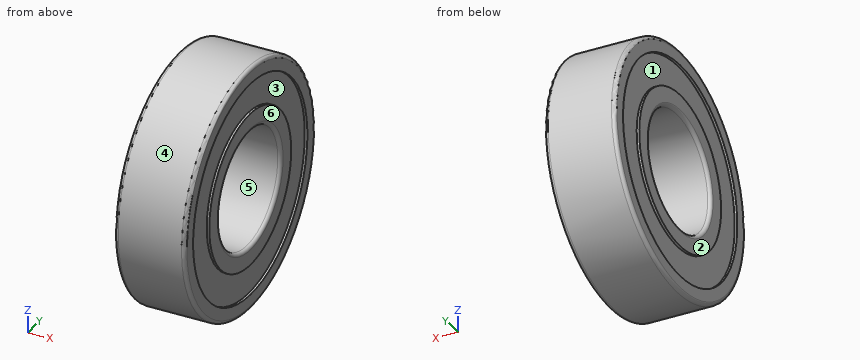
```python
from build123d import *


with BuildPart() as part:
    # 草图1 → 旋转1 (revolve)
    with BuildSketch(Plane.XY, mode=Mode.PRIVATE) as revolve_1_sk:
        with BuildLine():
            Line((0, 20.4), (0, 18.4))
            Line((0, 18.4), (0.433, 18.4))
            Line((0.433, 18.4), (0.433, 13.2))
            Line((0.433, 13.2), (0, 13.2))
            Line((0, 13.2), (0, 10.6))
            ThreePointArc((0, 10.6), (0.175735931, 10.175735931), (0.6, 10))
            Line((0.6, 10), (11.4, 10))
            ThreePointArc((11.4, 10), (11.824264069, 10.175735931), (12, 10.6))
            Line((12, 10.6), (12, 13.2))
            Line((12, 13.2), (11.567, 13.2))
            Line((11.567, 13.2), (11.567, 18.4))
            Line((11.567, 18.4), (12, 18.4))
            Line((12, 18.4), (12, 20.4))
            ThreePointArc((12, 20.4), (11.824264069, 20.824264069), (11.4, 21))
            Line((11.4, 21), (0.6, 21))
            ThreePointArc((0.6, 21), (0.175735931, 20.824264069), (0, 20.4))
        make_face()
    revolve(revolve_1_sk.sketch.rotate(Axis((12, 0, 0), (-1, 0, 0)), 270), axis=Axis((12, 0, 0), (-1, 0, 0)))


solid = part.part
```
Input: part model. Units: mm. Frame: model coordinates. Face numbers are marked on the shaded views. A direction names the side the tool comes from. Coordinates: 2 decimals unless noted, no trailing zeros. Order: outer loops, then holes, each group sorted by start corner. A loop starts at its lowest first (then second) coordinate and runs counter-clockwise, first axis right, second up. Notation, with made-up numbers: (33, -27) - (49, -27) arc R23 ccw to (49, -17) - close; hole circle Ø7 at (-18, 18). An arc over 180 degrees is marked (long way). Return JSON: item names as keys, results as strings.
Q1. Cut plane C-C (x = 5). Return loops of the section in (y, z).
The answers:
{"outline": "circle Ø42 at (0, 0); hole circle Ø20 at (0, 0)"}
Q2. First-contact query: pin 1 (1.5 mm diameter, centred on x = 10.5, y = -15.5, fed in from +Z); pin 2 (1.5 mm diameter, centred on x = 2, y = 11, fed in from +Z); pin 3 (4 mm diameter, centred on y = -4, z = 16.5, fed in from -X); pin 4 (4 mm diameter, centred on x = 1.5, z = 8, fed in from -Y). Flat tips, straight axial feed; report the tip coordinate or a pass-through.
The answers:
{"pin 1": "stops at z = 14.95", "pin 2": "stops at z = 18.33", "pin 3": "stops at x = 0", "pin 4": "stops at y = -20.12"}
Q3. Draft query along Z for the marked faces 4, 5 and 6. Return one class per face: +Z half, -Z half, draft (parallel to the pull), parting line (faces both ways), or undercut.
The answers:
{"face 4": "parting line", "face 5": "undercut", "face 6": "draft"}
Q4. Ray query, probe 1 along Y at (x, z) = (11.75, -4); probe 2 along Y at (x, z) = (11.7, 0); probe 3 along Y at (x, z) = (3.5, 0). Return the intervals inside material, ascending.
The answers:
{"probe 1": "y = -20.5 to -17.96, -12.58 to -9.29, 9.29 to 12.58, 17.96 to 20.5", "probe 2": "y = -20.92 to -18.4, -13.2 to -10.08, 10.08 to 13.2, 18.4 to 20.92", "probe 3": "y = -21 to -10, 10 to 21"}
Q5. Access query for the marked faces 1, 2 and 3. Directions: +Z, -Z, +X, -X, +Y, -Y. A direction counts if a zero-diameter tool reaches every point of the face in a straight line with its end or side. Return the directions, or none.
The answers:
{"face 1": "-X", "face 2": "+Z, -Z, -X, +Y, -Y", "face 3": "+X"}
